from build123d import *

# Parameters (mm, degrees)
SKETCH_3_W          = 58
SKETCH_3_H          = 58
CUT_EXTRUDE_1_DEPTH = 7
SCALE_1_SCALE       = 0.5


with BuildPart() as part:
    # 草图1 → 旋转1 (revolve)
    with BuildSketch(Plane.XY, mode=Mode.PRIVATE) as revolve_1_sk:
        Polygon((0, 0), (0, 14.5), (1.154700538, 16.5), (6.5, 16.5), (6.5, 14.2), (7, 14.2), (7, 0), align=None)
    revolve(revolve_1_sk.sketch.rotate(Axis((7, 0, 0), (-1, 0, 0)), 270), axis=Axis((7, 0, 0), (-1, 0, 0)))

    # 草图2 → 切除-旋转1 (revolve, cut)
    with BuildSketch(Plane.XY, mode=Mode.PRIVATE) as cut_revolve_1_sk:
        Polygon((0, 0), (0, 11), (0.812, 10.188), (6.188, 10.188), (7, 11), (7, 0), align=None)
    revolve(cut_revolve_1_sk.sketch.rotate(Axis((7, 0, 0), (-1, 0, 0)), 270), axis=Axis((7, 0, 0), (-1, 0, 0)), mode=Mode.SUBTRACT)

    # 草图3 → 切除-拉伸1 (cut)
    with BuildSketch(Plane(origin=(0, 0, 0), x_dir=(0, 0, -1), z_dir=(1, 0, 0))):
        Rectangle(SKETCH_3_W, SKETCH_3_H)
        Polygon((-14.5, -8.371578903), (0, -16.743157806), (14.5, -8.371578903), (14.5, 8.371578903), (0, 16.743157806), (-14.5, 8.371578903), align=None, mode=Mode.SUBTRACT)
    extrude(amount=CUT_EXTRUDE_1_DEPTH, mode=Mode.SUBTRACT)


with BuildPart() as part_1:
    # 缩放比例1: scaled about (3.473718043, 0, 0)
    add(part.part.scale(SCALE_1_SCALE).moved(Location((1.736859021, 0, 0))))


solid = part_1.part
Source: CAD feature listing. Evaluate the final solid. Frame: model axes, mm. A direction names the side the tool comes from. Coordinates: 2 decimals unless noted, no trailing zeros. Loops run counter-clockwise (first coordinate to the right, second up) from the corner with the lowest first, then second, coordinate; pieces in that order, holes last. Notation, with made-up numbers: (-22, 6.5) - (-2, 6.5) arc R12 cw to (-2, 17.5) - close; hole circle Ø7 at (-37.75, 82). An arc over 180 degrees is marked (long way). One line per item, written item: value. Start each with the question number.
1. Set-up query: faces 1 (the flat face through (3.339, -6.306, -3.577)), 2 (the flat face through (4.987, 7, -2)). Return all of +Z, -Z, +X, -X, +Y, -Y with unobstructed straight access to the full face (end or side cutting, diameter ignored); none if empty.
2. Contact query for flat-ended pins moving along their axis: P1, Ø2, axis at x = 3, y = 6, coming from the -Z side; P2, Ø6, axis at y = 0, z = 0, coming from the -X side; P3, Ø1.5, axis at x = 2, z = -3.5, coming from the +Y side; P4, Ø1.5, axis at x = 3, z = -5, coming from the +Y side. Output: stop coordinate, or through.
3. Ray query, L1, parallel to Y at x = 4.2, z = 0; L2, parallel to Y at x = 4.8, z = 0.5; L3, parallel to Z at x = 4.95, y = 1.5. Return the intervals inside material, ascending.
4. Section B-B (z = 0). Return the cut outline in (x, y).
5. Section A-A (x = 3.95). Return the cut outline in (y, z), and give its area (3 significant figures).
6. Mould query, pull axis Y, two halves, no side actions, for faces 3 (the cylindrical face through (3.51, 1.53, 4.86)), 4 (the flat face through (3.339, 6.251, -3.673)), 5 (the flat face through (3, 0, -7.25)), 6 (the conical face through (1.9, -7.53, -0.02)). Classes: pulls with the +Y half, pulls with the -Y half, needs draft (parallel to the pull), parting line crosses it, or undercut.
Verdict:
1. face 1: -Z, +X, -X, -Y
1. face 2: +X
2. P1: stops at z = -5.84
2. P2: passes through
2. P3: stops at y = 6.78
2. P4: stops at y = 5.92
3. L1: y = -8.25 to -5.09, 5.09 to 8.25
3. L2: y = -8.08 to -5.07, 5.07 to 8.08
3. L3: z = -7.25 to -4.99, 4.99 to 7.25
4. outline: (1.74, -7.25) - (2.31, -8.25) - (4.99, -8.25) - (4.99, -7.1) - (5.24, -7.1) - (5.24, -5.5) - (4.83, -5.09) - (2.14, -5.09) - (1.74, -5.5) - close; (1.74, 5.5) - (2.14, 5.09) - (4.83, 5.09) - (5.24, 5.5) - (5.24, 7.1) - (4.99, 7.1) - (4.99, 8.25) - (2.31, 8.25) - (1.74, 7.25) - close
5. outline: (-8.25, -0.22) - (-4.31, -7.03) arc R8.25 ccw to (-3.94, -7.25) - (3.94, -7.25) arc R8.25 ccw to (4.31, -7.03) - (8.25, -0.22) arc R8.25 ccw to (8.25, 0.22) - (4.31, 7.03) arc R8.25 ccw to (3.94, 7.25) - (-3.94, 7.25) arc R8.25 ccw to (-4.31, 7.03) - (-8.25, 0.22) arc R8.25 ccw to start; hole circle Ø10.19 at (0, 0)
5. area: 100 mm2
6. face 3: undercut
6. face 4: pulls with the +Y half
6. face 5: needs draft
6. face 6: pulls with the -Y half
